Geometry: see drawing. Coordinates: mm, zero at the bounding-box minimum. A direction names the side the tool comes from. Round coordinates to 2 decimals unless told otherwise and drop trailing zeros. Loops run counter-clockwise (first coordinate to the right, second up) from the corner with the lowest first, then second, coordinate; pieces in that order, holes last.
(1) Mould query, pull axis X, two halves, no side actions, for the marked faces 4, 5, 6 and 7. Classes: pulls with the +X half, pulls with the -X half, needs draft (parallel to the pull), parting line crosses it, or undercut.
(2) Section C-C, the plane z = 10. Return the cut outline in (x, y).
(3) Material intervals for probe 1 along X at (y, z) = (13.5, 10); probe 2 along Z at (x, y) = (10, 37); probe 3 along X at (y, z) = (24, 9), sorted ascending.
(4) First-contact query: pin 1 Ø3 at (x, z) = (42, 6) entering from +Y; pin 2 Ø11.5 at (x, z) = (30, 10) entering from -Y; pin 3 Ø2 at (x, z) = (43, 15) entering from -Y; pin 4 Ø2 at (y, z) = (45, 9.5) entering from +X. Flat tips, straight axial feed; report the tip coordinate or a pass-through.
(5) Section A-A, the plane x = 30. Return the cut outline in (y, z).
(6) Section D-D, the plane x = 4. Return the cut outline in (y, z), plus the area to 3 significant figures.
(7) Set-up query: the marked faces 1, 2 and 3. Return all of +Z, -Z, +X, -X, +Y, -Y with unobstructed straight access to the full face (end or side cutting, diameter ignored); none if empty.
(8) Section B-B, the plane y = 23.5. Return the cut outline in (x, z).
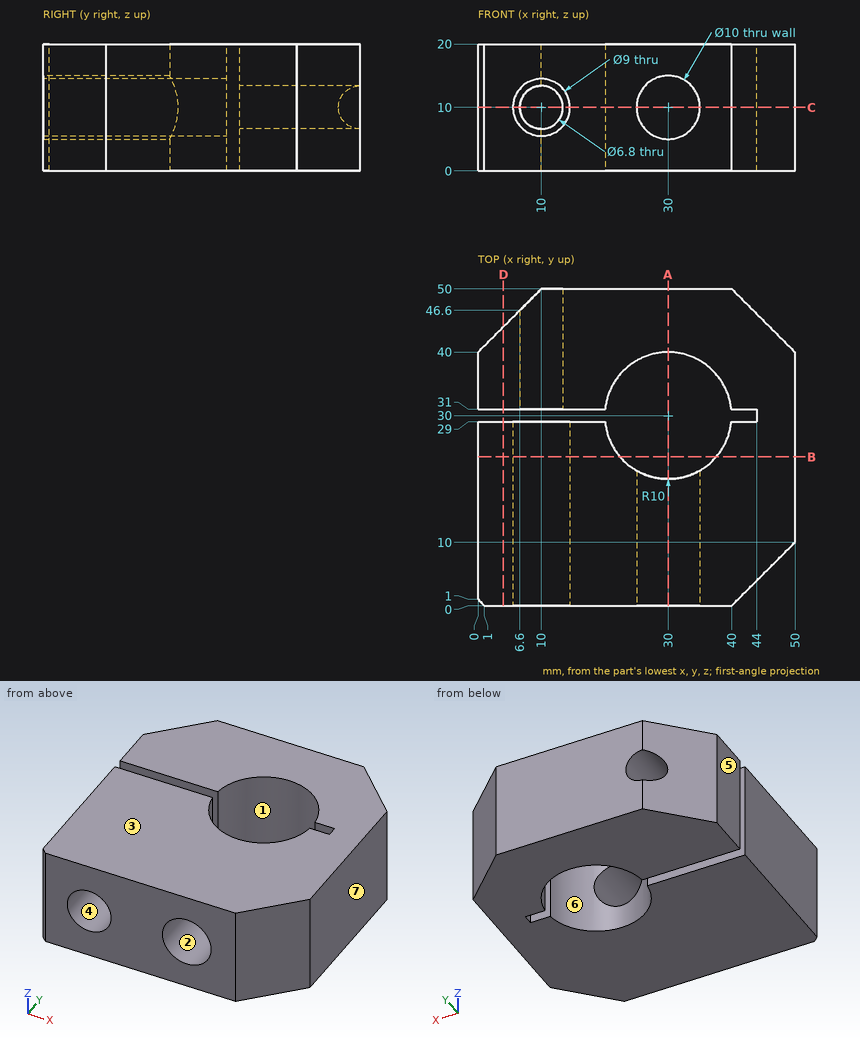
Output values:
1. face 4: undercut
1. face 5: pulls with the -X half
1. face 6: undercut
1. face 7: pulls with the +X half
2. outline: (0, 1) - (1, 0) - (5.5, 0) - (5.5, 29) - (0, 29) - close; (0, 31) - (6.6, 31) - (6.6, 46.6) - (0, 40) - close; (13.4, 31) - (20.05, 31) arc R10 cw to (39.95, 31) - (44, 31) - (44, 29) - (39.95, 29) arc R10 cw to (35, 21.34) - (35, 0) - (40, 0) - (50, 10) - (50, 40) - (40, 50) - (13.4, 50) - close; (14.5, 0) - (25, 0) - (25, 21.34) arc R10 cw to (20.05, 29) - (14.5, 29) - close
3. probe 1: x = 0 to 5.5, 14.5 to 25, 35 to 50
3. probe 2: z = 0 to 6.6, 13.4 to 20
3. probe 3: x = 0 to 5.61, 14.39 to 22, 38 to 50
4. pin 1: stops at y = 49.5
4. pin 2: stops at y = 0
4. pin 3: stops at y = 2
4. pin 4: stops at x = 46
5. outline: (0, 0) - (20, 0) - (20, 5) - (0, 5) - close; (0, 15) - (20, 15) - (20, 20) - (0, 20) - close; (40, 0) - (50, 0) - (50, 20) - (40, 20) - close
6. outline: (0, 0) - (29, 0) - (29, 20) - (0, 20) - close; (31, 0) - (44, 0) - (44, 20) - (31, 20) - close
6. area: 840 mm2
7. face 1: +Z, -Z
7. face 2: -Y
7. face 3: +Z, +X, -X, +Y, -Y
8. outline: (0, 0) - (22.4, 0) - (22.4, 20) - (0, 20) - close; (37.6, 0) - (50, 0) - (50, 20) - (37.6, 20) - close; hole circle Ø9 at (10, 10)
